The drawing under review shows one solid part. Ordinate dimensions are in mm from its lowest x, y, z. Round coordinates to 2 decimals unless told otherwise and drop trailing zeros. Loops run counter-clockwise (first coordinate to the right, second up) from the corner with the lowest first, then second, coordinate; pieces in that order, holes last. Notation, with made-up numbers: M 61.5,27.5 L 89.5,27.5 A8 ccw 89.5,40.5 Z; hole C 72.5,36 d5. An arc over 180 degrees is marked long. Use a Markdown table: item, result.
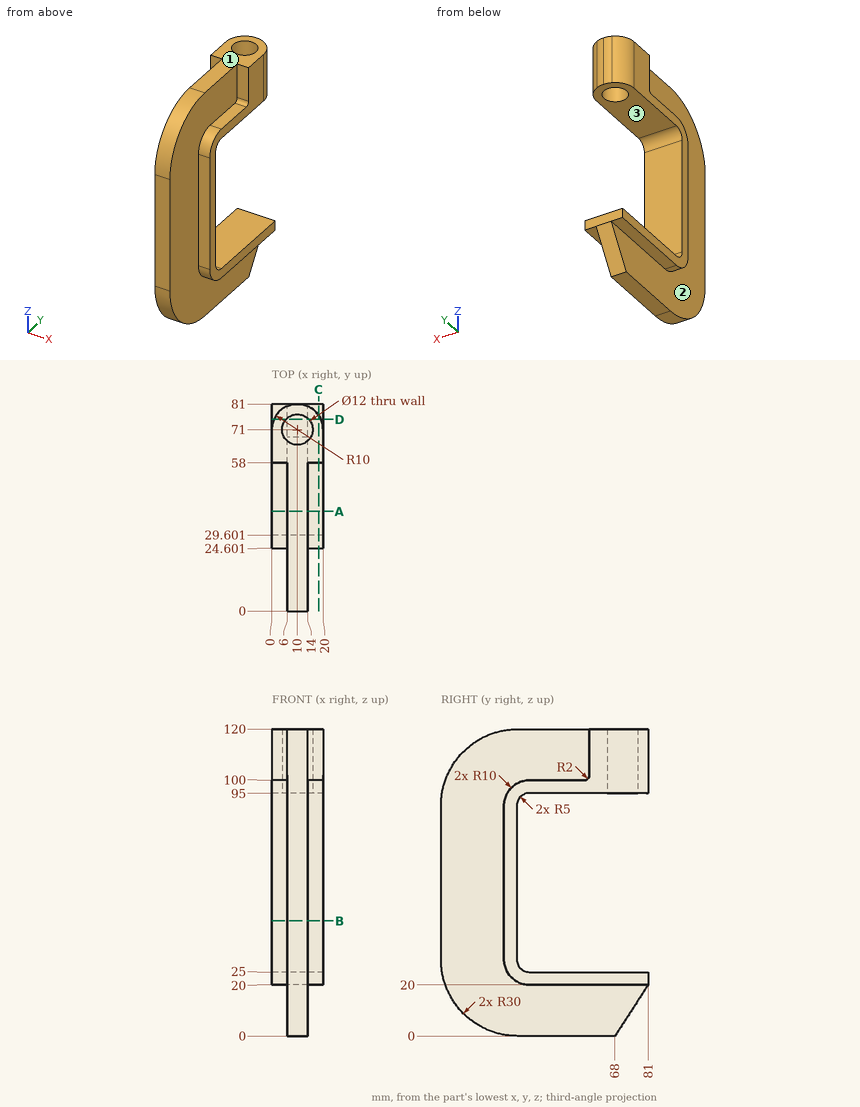
1. Take a section at A-A on y = 39. Give the boundary of the cut face in (x, z), and give its area (3 significant figures).
Check values:
| item | result |
|---|---|
| outline | M 0,20 L 6,20 L 6,0 L 14,0 L 14,20 L 20,20 L 20,25 L 0,25 Z; M 0,95 L 20,95 L 20,100 L 14,100 L 14,120 L 6,120 L 6,100 L 0,100 Z |
| area | 520 mm² |
2. Take a section at D-D on y = 75. Give the boundary of the cut face in (x, z) (1 decimal).
Check values:
| item | result |
|---|---|
| outline | M 0,20 L 6,20 L 6,10.8 L 14,10.8 L 14,20 L 20,20 L 20,25 L 0,25 Z; M 0.8,95 L 5.5,95 L 5.5,120 L 0.8,120 Z; M 14.5,95 L 19.2,95 L 19.2,120 L 14.5,120 Z |
3. Wall thickness on line 1 along Z through (x, y) = (8.5, 64); line 2 along Z through (x, y) = (2, 47); line 3 along X through (y, z) = (5, 81): over which ranges is each line inside the solid? List them lowest first. Write a range as from..to.
Check values:
| item | result |
|---|---|
| line 1 | z = 0..25, 95..120 |
| line 2 | z = 20..25, 95..100 |
| line 3 | x = 6..14 |
4. Take a section at B-B on z = 45. Give the boundary of the cut face in (x, y).
Check values:
| item | result |
|---|---|
| outline | M 0,24.6 L 6,24.6 L 6,0 L 14,0 L 14,24.6 L 20,24.6 L 20,29.6 L 0,29.6 Z |
5. Take a section at C-C on x = 18.25. Give the boundary of the cut face in (y, z), and give its area (3 significant figures).
Check values:
| item | result |
|---|---|
| outline | M 24.6,30 A10 ccw 34.6,20 L 81,20 L 81,25 L 34.6,25 A5 cw 29.6,30 L 29.6,90 A5 cw 34.6,95 L 76.65,95 L 76.65,120 L 58,120 L 58,102 A2 cw 56,100 L 34.6,100 A10 ccw 24.6,90 Z |
| area | 1,230 mm² |
6. The part is to be moulded in two halves that separate along Z. For the marked faces 1, 2 and 3, say which applies: pulls with the +Z half, pulls with the -Z half, needs draft (parallel to the pull), parting line crosses it, or undercut.
Check values:
| item | result |
|---|---|
| face 1 | pulls with the +Z half |
| face 2 | needs draft |
| face 3 | undercut |
7. Insertion check: pin 1 (3 mm diameter, centred on x = 3.5, y = 62, fed in from -Z); pin 2 (3 mm diameter, centred on x = 7, y = 45, fed in from -Z); pin 3 (3 mm diameter, centred on x = 2, y = 47, fed in from +Z); pin 4 (9.5 mm diameter, centred on x = 10, y = 71, fed in from +Z). Each pin has a flat end and moves straight along its axis. Give the tip position at first contact, or say it passes through.
Check values:
| item | result |
|---|---|
| pin 1 | stops at z = 20 |
| pin 2 | stops at z = 0 |
| pin 3 | stops at z = 100 |
| pin 4 | stops at z = 25 |
